Geometry: final body of the model. Coordinates: model frame, mm. A direction names the side the tool comes from. Round coordinates to 2 decimals unless told otherwise and drop trailing zeros. Write each loop counter-clockwise with the first axis right and the second up, starting at its lowest first coordinate (ties: lowest second). Pieces come first, ordered by that corner, then holes. Notation, with made-up numbers: (3, -5) - (7, -5) arc R21 cw to (7, 1) - close; hole circle Ø1 at (66, 63). An arc over 180 degrees is marked (long way). Use a Markdown table: item, result. Add a question column.
```python
from build123d import *

# Parameters (mm, degrees)
SKETCH_1_W                = 125
SKETCH_1_H                = 156
EXTRUDE_1_DEPTH           = 12
SKETCH_2_W                = 55
SKETCH_2_H                = 36
CUT_EXTRUDE_1_DEPTH       = 101.669012114
SKETCH_3_W                = 70
SKETCH_3_H                = 35
CUT_EXTRUDE_2_DEPTH       = 3
HOLE_WIZARD_1_D           = 5.5
HOLE_WIZARD_1_CBORE_D     = 10
HOLE_WIZARD_1_CBORE_DEPTH = 5.7
HOLE_WIZARD_2_D           = 6.6
HOLE_WIZARD_2_CBORE_D     = 11
HOLE_WIZARD_2_CBORE_DEPTH = 6.8
CHAMFER_1_SIZE            = 2
FILLET_1_R                = 1
SKETCH_10_R               = 25
CUT_EXTRUDE_3_DEPTH       = 101.669012114
HOLE_WIZARD_M5_1_D        = 4.2
HOLE_WIZARD_M4_1_D        = 3.3


with BuildPart() as part:
    # 草图1 → 凸台-拉伸1 (new body)
    with BuildSketch(Plane.XY):
        Rectangle(SKETCH_1_W, SKETCH_1_H)
    extrude(amount=EXTRUDE_1_DEPTH)

    # 草图2 → 切除-拉伸1 (cut, through all)
    with BuildSketch(Plane.XY.offset(12)):
        with Locations((-35, 60)):
            Rectangle(SKETCH_2_W, SKETCH_2_H)
    extrude(amount=-CUT_EXTRUDE_1_DEPTH, mode=Mode.SUBTRACT)

    # 草图3 → 切除-拉伸2 (cut)
    with BuildSketch(Plane(origin=(0, 0, 0), x_dir=(-1, 0, 0), z_dir=(0, 0, -1))):
        with Locations((-27.5, 60.5)):
            Rectangle(SKETCH_3_W, SKETCH_3_H)
    extrude(amount=-CUT_EXTRUDE_2_DEPTH, mode=Mode.SUBTRACT)

    # 打孔尺寸(%根据)内六角圆柱头螺钉的类型1 (through all)
    with Locations(Plane(origin=(0, 0, 0), x_dir=(-1, 0, 0), z_dir=(0, 0, -1))):
        with Locations((-55, -72), (0, -72), (55, -72)):
            CounterBoreHole(HOLE_WIZARD_1_D / 2, HOLE_WIZARD_1_CBORE_D / 2, HOLE_WIZARD_1_CBORE_DEPTH)

    # 打孔尺寸(%根据)内六角圆柱头螺钉的类型2 (through all)
    with Locations(Plane(origin=(0, 0, 12), x_dir=(-1, 0, 0), z_dir=(0, 0, 1))):
        with Locations((-52.5, -63), (-27.5, -63), (-2.5, -63)):
            CounterBoreHole(HOLE_WIZARD_2_D / 2, HOLE_WIZARD_2_CBORE_D / 2, HOLE_WIZARD_2_CBORE_DEPTH)

    # 倒角1
    chamfer_1_edges = [part.edges().sort_by_distance(p)[0] for p in [
        (-62.5, 42, 6),
        (-7.5, 78, 7.5),
        (62.5, -78, 6),
        (-62.5, -78, 6),
        (62.5, 78, 7.5),
    ]]
    chamfer(chamfer_1_edges, length=CHAMFER_1_SIZE)

    # 圆角1
    fillet_1_edges = [part.edges().sort_by_distance(p)[0] for p in [
        (-7.5, 42, 6),
    ]]
    fillet(fillet_1_edges, radius=FILLET_1_R)

    # 草图10 → 切除-拉伸3 (cut, through all)
    with BuildSketch(Plane.XY.offset(12)):
        with Locations((0, -28)):
            Circle(SKETCH_10_R)
    extrude(amount=-CUT_EXTRUDE_3_DEPTH, mode=Mode.SUBTRACT)

    # M5 螺纹孔1 (through all)
    with Locations(Plane(origin=(0, 0, 0), x_dir=(-1, 0, 0), z_dir=(0, 0, -1))):
        with Locations((-23.55, -4.45), (23.55, -4.45), (23.55, -51.55), (-23.55, -51.55)):
            Hole(HOLE_WIZARD_M5_1_D / 2)

    # M4 螺纹孔1 (through all)
    with Locations(Plane.XY.offset(12)):
        with Locations((2.053366632, 9.443740271), (-36.520933317, -36.513015309)):
            Hole(HOLE_WIZARD_M4_1_D / 2)


solid = part.part
```
1) Pin query (flat end, axial travel): P1, Ø3.5, axis at x = 0.5, y = 61, coming from the +Z side; P2, Ø3, axis at x = -36.52, y = -36.51, coming from the +Z side; P3, Ø4, axis at x = -14.5, z = 2.5, coming from the +Y side; P4, Ø3, axis at x = -55, y = -73.5, coming from the -Z side. Return the tip coordinate at first contact, or that it passes through.
2) Material intervals for L1, parallel to X at y = 63, z = 10.25; L2, parallel to Y at x = -55, z = 4.55; L3, parallel to X at y = 67, z = 8.75, sorted ascending. Write a range as from..to.
3) Set-up query: faces 1 (the cylindrical face through (-25.65, -4.36, 6.08)), 2 (the flat face through (-2.2, -74.2, 5.7)), 3 (the flat face through (53, 67, 5.2)). Return all of +Z, -Z, +X, -X, +Y, -Y with unobstructed straight access to the full face (end or side cutting, diameter ignored); none if empty.
4) Section B-B, the plane z = 9. State how many separate pieces and enclosed holes the cut face has, then the cut area to 3 significant figures.
5) Section C-C, the plane x = -55. Return the cut outline in (y, z), then the cut area to 3 significant figures.
6) Section D-D, the plane y = 46.5. Return the cut outline in (x, z).
7) Draft query along X for faces 4 (the cylindrical face through (50.07, 60.77, 4.08)), 5 (the flat face through (-57.2, -74.2, 5.7)), 6 (the flat face through (-35, 42, 6)). Return one class per face: released by +X, released by -X, zero draft, split by the parting line, or undercut.
8) Section A-A, the plane x = 27.5. Return the cut outline in (y, z).
Output values:
| question | item | result |
|---|---|---|
| 1 | P1 | stops at z = 5.2 |
| 1 | P2 | passes through |
| 1 | P3 | stops at y = 42 |
| 1 | P4 | stops at z = 5.7 |
| 2 | L1 | x = -7.5..-3, 8..22, 33..47, 58..62.5 |
| 2 | L2 | y = -78..-77, -67..42 |
| 2 | L3 | x = -7.5..-1.27, 6.27..23.73, 31.27..48.73, 56.27..62.5 |
| 3 | face 1 | +Z, -Z |
| 3 | face 2 | -Z |
| 3 | face 3 | +Z |
| 4 | separate pieces | 1 |
| 4 | enclosed holes | 13 |
| 4 | area | 15,100 mm^2 |
| 5 | outline | (-78, 0) - (-77, 0) - (-77, 5.7) - (-74.75, 5.7) - (-74.75, 12) - (-78, 12) - close; (-69.25, 5.7) - (-67, 5.7) - (-67, 0) - (42, 0) - (42, 12) - (-69.25, 12) - close |
| 5 | area | 1,350 mm^2 |
| 6 | outline | (-7.5, 3) - (62.5, 3) - (62.5, 12) - (-7.5, 12) - close |
| 7 | face 4 | undercut |
| 7 | face 5 | undercut |
| 7 | face 6 | zero draft |
| 8 | outline | (-78, 0) - (43, 0) - (43, 3) - (59.7, 3) - (59.7, 5.2) - (57.5, 5.2) - (57.5, 12) - (-78, 12) - close; (66.3, 3) - (78, 3) - (78, 12) - (68.5, 12) - (68.5, 5.2) - (66.3, 5.2) - close |
